The listing builds one solid part. Answer for the finished solid, in the listing's coordinates (mm). Face numbers are marked on the shaded views. Coordinates: 2 decimals unless noted, no trailing zeros. Order: outer loops, then holes, each group sorted by start corner. A loop starts at its lowest first (then second) coordinate and runs counter-clockwise, first axis right, second up. Notation, with made-up numbers: (-28.75, 46) -> (11.25, 46) arc R16 cw to (11.25, 68) -> close; hole circle Ø2 at (40, 57.25). An arc over 180 degrees is marked (long way). Return JSON: item names as keys, results as strings.
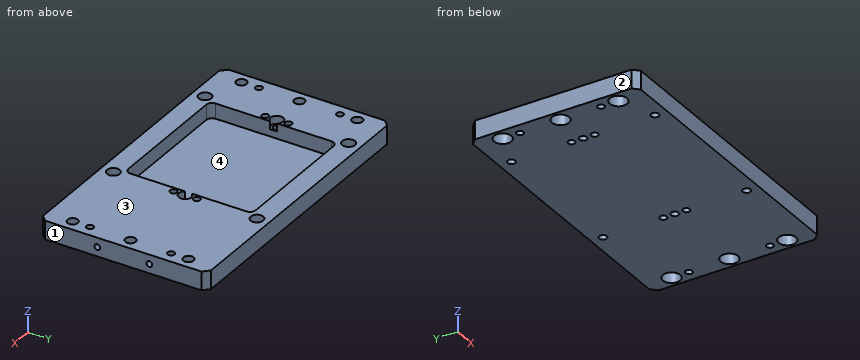
```python
from build123d import *

# Parameters (mm, degrees)
SKETCH_1_W                  = 252
SKETCH_1_H                  = 145
EXTRUDE_1_DEPTH             = 8
HOLE_WIZARD_2_D             = 6.6
HOLE_WIZARD_2_CBORE_D       = 11
HOLE_WIZARD_2_CBORE_DEPTH   = 6.8
HOLE_WIZARD_2_2_D           = 9
HOLE_WIZARD_2_2_CBORE_D     = 15
HOLE_WIZARD_2_2_CBORE_DEPTH = 9
HOLE_WIZARD_6_0_6_1_D       = 6
HOLE_WIZARD_6_0_6_2_D       = 6
CUT_EXTRUDE_1_DEPTH         = 13
CHAMFER_1_SIZE              = 5
HOLE_WIZARD_M6_2_D          = 5
HOLE_WIZARD_M6_2_DEPTH      = 23
HOLE_WIZARD_M6_2_TIP        = 1.502151548


with BuildPart() as part:
    # 草图1 → 凸台-拉伸1 (new, symmetric)
    with BuildSketch(Plane.XY):
        Rectangle(SKETCH_1_W, SKETCH_1_H)
    extrude(amount=EXTRUDE_1_DEPTH, both=True)

    # Hole Wizard 2 (through all)
    with Locations(Plane.XY.offset(8)):
        with Locations((-85, 62), (-85, 0), (41, 62), (41, 0), (41, -62), (-85, -62)):
            CounterBoreHole(HOLE_WIZARD_2_D / 2, HOLE_WIZARD_2_CBORE_D / 2, HOLE_WIZARD_2_CBORE_DEPTH)

    # Hole Wizard 2 2 (through all)
    with Locations(Plane(origin=(0, 0, -8), x_dir=(-1, 0, 0), z_dir=(0, 0, -1))):
        with Locations((-116, -50), (-116, 0), (-116, 50)):
            hole_wizard_2_2 = CounterBoreHole(HOLE_WIZARD_2_2_D / 2, HOLE_WIZARD_2_2_CBORE_D / 2, HOLE_WIZARD_2_2_CBORE_DEPTH)

    # Ø6.0 (6) 直径孔1 (through all)
    with Locations(Plane(origin=(0, 0, -8), x_dir=(-1, 0, 0), z_dir=(0, 0, -1))):
        with Locations((-116, -35), (-116, 35)):
            hole_wizard_6_0_6_1 = Hole(HOLE_WIZARD_6_0_6_1_D / 2)

    # 镜向1: Hole Wizard 2 2, Ø6.0 (6) 直径孔1 across plane
    add(hole_wizard_2_2.mirror(Plane(origin=(0, 0, 0), x_dir=(0, 0, 1), z_dir=(1, 0, 0))), mode=Mode.SUBTRACT)
    add(hole_wizard_6_0_6_1.mirror(Plane(origin=(0, 0, 0), x_dir=(0, 0, 1), z_dir=(1, 0, 0))), mode=Mode.SUBTRACT)

    # Ø6.0 (6) 直径孔2 (through all)
    with Locations(Plane.XY.offset(8)):
        with Locations((41, -10), (-85, -10), (-85, 10), (41, 10)):
            Hole(HOLE_WIZARD_6_0_6_2_D / 2)

    # 草图10 → 切除-拉伸1 (cut)
    with BuildSketch(Plane.XY.offset(8)):
        with BuildLine():
            Line((-75.5, 55), (31.5, 55))
            ThreePointArc((31.5, 55), (35.035533906, 53.535533906), (36.5, 50))
            Line((36.5, 50), (36.5, -50))
            ThreePointArc((36.5, -50), (35.035533906, -53.535533906), (31.5, -55))
            Line((31.5, -55), (-75.5, -55))
            ThreePointArc((-75.5, -55), (-79.035533906, -53.535533906), (-80.5, -50))
            Line((-80.5, -50), (-80.5, 50))
            ThreePointArc((-80.5, 50), (-79.035533906, 53.535533906), (-75.5, 55))
        make_face()
    extrude(amount=-CUT_EXTRUDE_1_DEPTH, mode=Mode.SUBTRACT)

    # 倒角1
    chamfer_1_edges = [part.edges().sort_by_distance(p)[0] for p in [
        (-126, 72.5, 0),
        (126, 72.5, 0),
        (126, -72.5, 0),
        (-126, -72.5, 0),
    ]]
    chamfer(chamfer_1_edges, length=CHAMFER_1_SIZE)

    # M6 螺纹孔2
    with Locations(Plane(origin=(126, 0, 0), x_dir=(0, 0, -1), z_dir=(1, 0, 0))):
        with Locations((0, 22.5), (0, -22.5)):
            Hole(HOLE_WIZARD_M6_2_D / 2, depth=HOLE_WIZARD_M6_2_DEPTH)
            with Locations((0, 0, -(HOLE_WIZARD_M6_2_DEPTH + HOLE_WIZARD_M6_2_TIP / 2))):  # 118° drill point
                Cone(0, HOLE_WIZARD_M6_2_D / 2, HOLE_WIZARD_M6_2_TIP, mode=Mode.SUBTRACT)


solid = part.part
```
Item 1: The part is cut by section D-D on y = -10. Determine the outline of the cut face in (x, z).
Answer list:
{"outline": "(-126, -8) -> (-88, -8) -> (-88, 8) -> (-126, 8) -> close; (-82, -8) -> (38, -8) -> (38, 8) -> (36.5, 8) -> (36.5, -5) -> (-80.5, -5) -> (-80.5, 8) -> (-82, 8) -> close; (44, -8) -> (126, -8) -> (126, 8) -> (44, 8) -> close"}
Item 2: Find the intervals of material crossed by probe 1 along Y at (x, z) = (-116, -2.25); probe 2 along X at (y, z) = (-56, -4); probe 3 along Y at (x, z) = (-116, 6.25), in increasing order.
Answer list:
{"probe 1": "-72.5 to -57.5, -42.5 to -38, -32 to -7.5, 7.5 to 32, 38 to 42.5, 57.5 to 72.5", "probe 2": "-126 to -120.5, -111.5 to 111.5, 120.5 to 126", "probe 3": "-72.5 to -54.5, -45.5 to -38, -32 to -4.5, 4.5 to 32, 38 to 45.5, 54.5 to 72.5"}
Item 3: The part is cut by section C-C on x = 116. Count the separate pieces of the cut face and the enclosed holes in it, plus the area to 3 significant figures.
Answer list:
{"separate pieces": "6", "enclosed holes": "2", "area": "1,490 mm2"}
Item 4: Determine the mould class of the marked faces 1, 2, 3 and 4 for opening direction X: pulls with the +X half, pulls with the -X half, needs draft (parallel to the pull), parting line crosses it, or undercut.
Answer list:
{"face 1": "pulls with the +X half", "face 2": "pulls with the -X half", "face 3": "needs draft", "face 4": "undercut"}
Item 5: The part is cut by section B-B on x = -68. Determine the outline of the cut face in (y, z).
Answer list:
{"outline": "(-72.5, -8) -> (72.5, -8) -> (72.5, 8) -> (55, 8) -> (55, -5) -> (-55, -5) -> (-55, 8) -> (-72.5, 8) -> close"}
Item 6: Flat-ended cylindrical pins translate along their axes: pin 1 (4.5 mm diameter, centred on x = -119, y = -50, fed in from -Z); pin 2 (8.5 mm diameter, centred on x = -85, y = -62, fed in from +Z). Find the tip coordinate at first contact, or state that the pin passes through.
Answer list:
{"pin 1": "z = 1", "pin 2": "z = 1.2"}
Item 7: The part is cut by section A-A on y = -62. Determine the outline of the cut face in (x, z), plus the area to 3 significant figures.
Answer list:
{"outline": "(-126, -8) -> (-88.3, -8) -> (-88.3, 1.2) -> (-90.5, 1.2) -> (-90.5, 8) -> (-126, 8) -> close; (-81.7, -8) -> (37.7, -8) -> (37.7, 1.2) -> (35.5, 1.2) -> (35.5, 8) -> (-79.5, 8) -> (-79.5, 1.2) -> (-81.7, 1.2) -> close; (44.3, -8) -> (126, -8) -> (126, 8) -> (46.5, 8) -> (46.5, 1.2) -> (44.3, 1.2) -> close", "area": "3,760 mm2"}
